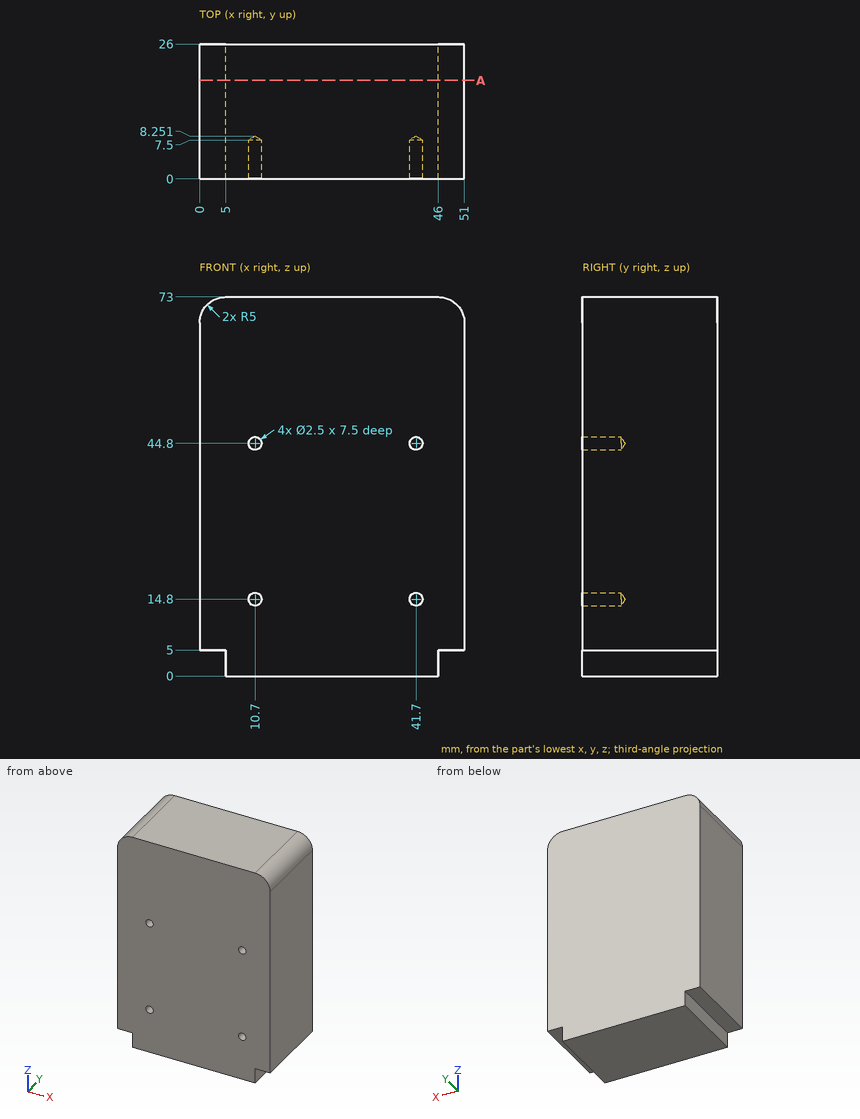
The drawing under review shows one solid part. Ordinate dimensions are in mm from its lowest x, y, z. Coordinates: 2 decimals unless noted, no trailing zeros. Write each loop counter-clockwise with the first axis right and the second up, starting at its lowest first coordinate (ties: lowest second). Pieces come first, ordered by that corner, then holes. Notation, with made-up numbers: M 17,41.25 L 62,41.25 A30 cw 62,72.25 Z; hole C 61.5,12.25 d2. An arc over 180 degrees is marked long. Put each result on its own line as item: value.
1) Clearance check with flat-ended pins moving along their axes: pin 1 Ø3 at (x, y) = (29.5, 17.5) entering from -Z; pin 2 Ø5.5 at (x, y) = (2, 17.5) entering from -Z; pin 3 Ø4 at (y, z) = (8.5, 1.5) entering from +X. State where each tip first meets the part, or that it passes through.
Computed:
pin 1: stops at z = 0
pin 2: stops at z = 5
pin 3: stops at x = 46
2) Add section A-A on y = 19. Give the boundary of the cut face in (x, z).
Computed:
outline: M 0,5 L 5,5 L 5,0 L 46,0 L 46,5 L 51,5 L 51,68 A5 ccw 46,73 L 5,73 A5 ccw 0,68 Z
3) Wall thickness on probe 1 along X at (y, z) = (4.5, 14.8); probe 2 along Z at (x, y) = (10.7, 1.5): over which ranges is each line inside the solid? List them lowest first. Write a range as [from, to].
Computed:
probe 1: x = [0, 9.45], [11.95, 40.45], [42.95, 51]
probe 2: z = [0, 13.55], [16.05, 43.55], [46.05, 73]
